Part model, mm, in its own coordinate system. Face numbers are marked on the shaded views. A direction names the side the tool comes from. Give positions to 0.01 mm unless a question says otherwise; leave off trailing zeros. Loops run counter-clockwise (first coordinate to the right, second up) from the corner with the lowest first, then second, coordinate; pieces in that order, holes last. Notation, with made-up numbers: (-27.75, 16.25) -> (-13.75, 16.25) arc R17 cw to (-13.75, 26.25) -> close; hole circle Ø4 at (-16.5, 81). An arc over 180 degrees is marked (long way). Write item = value, one per line.
from build123d import *

# Parameters (mm, degrees)
SKETCH1_W                                            = 110
SKETCH1_H                                            = 60
BOSS_EXTRUDE1_DEPTH                                  = 12
SKETCH2_R                                            = 12.5
CUT_EXTRUDE1_DEPTH                                   = 5
SKETCH3_R                                            = 10
CUT_EXTRUDE3_DEPTH                                   = 64.788713735
CHAMFER1_SIZE                                        = 3
M4_TAPPED_HOLE1_D                                    = 3.3
CBORE_FOR_M8_HEXAGON_SOCKET_HEAD_CAP_SCR_D           = 9
CBORE_FOR_M8_HEXAGON_SOCKET_HEAD_CAP_SCR_CBORE_D     = 15
CBORE_FOR_M8_HEXAGON_SOCKET_HEAD_CAP_SCR_CBORE_DEPTH = 9


with BuildPart() as part:
    # Sketch1 → Boss-Extrude1 (new body)
    with BuildSketch(Plane.XY):
        Rectangle(SKETCH1_W, SKETCH1_H)
    extrude(amount=BOSS_EXTRUDE1_DEPTH)

    # Sketch2 → Cut-Extrude1 (cut)
    with BuildSketch(Plane(origin=(0, 0, 12), x_dir=(-1, 0, 0), z_dir=(0, 0, -1))):
        with Locations((35, 0)):
            Circle(SKETCH2_R)
    extrude(amount=CUT_EXTRUDE1_DEPTH, mode=Mode.SUBTRACT)

    # Sketch3 → Cut-Extrude3 (cut, through all)
    with BuildSketch(Plane.XY.offset(12)):
        with Locations((-35, 0)):
            Circle(SKETCH3_R)
    extrude(amount=-CUT_EXTRUDE3_DEPTH, mode=Mode.SUBTRACT)

    # Chamfer1
    chamfer1_edges = [part.edges().sort_by_distance(p)[0] for p in [
        (55, -30, 6),
        (-55, -30, 6),
        (-55, 30, 6),
        (55, 30, 6),
    ]]
    chamfer(chamfer1_edges, length=CHAMFER1_SIZE)

    # M4 Tapped Hole1 (through all)
    with Locations(Plane.XY.offset(12)):
        with Locations((-35, 14.5), (-20.5, 0), (-49.5, 0), (-35, -14.5)):
            Hole(M4_TAPPED_HOLE1_D / 2)

    # CBORE for M8 Hexagon socket head cap screws1 (through all)
    with Locations(Plane(origin=(0, 0, 0), x_dir=(-1, 0, 0), z_dir=(0, 0, -1))):
        with Locations((-40, 15), (-40, -15)):
            CounterBoreHole(CBORE_FOR_M8_HEXAGON_SOCKET_HEAD_CAP_SCR_D / 2, CBORE_FOR_M8_HEXAGON_SOCKET_HEAD_CAP_SCR_CBORE_D / 2, CBORE_FOR_M8_HEXAGON_SOCKET_HEAD_CAP_SCR_CBORE_DEPTH)


solid = part.part
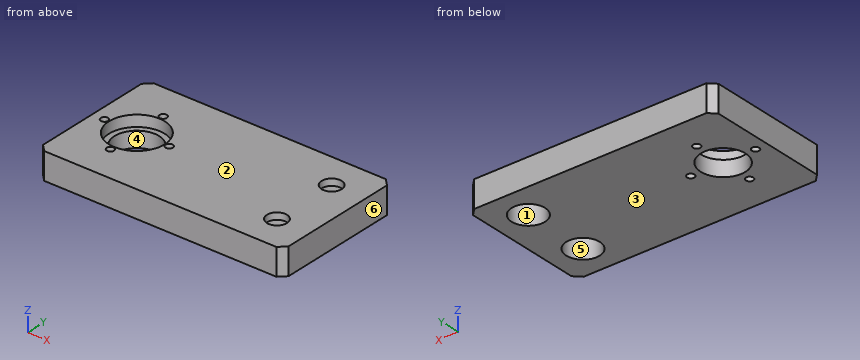
1) Slice it at C-C, the plane x = 42. List the corners of the cut face in (y, z).
Resolved:
outline = (-30, 0) -> (-22.23, 0) -> (-22.23, 9) -> (-19.03, 9) -> (-19.03, 12) -> (-30, 12) -> close; (-10.97, 9) -> (-7.77, 9) -> (-7.77, 0) -> (7.77, 0) -> (7.77, 9) -> (10.97, 9) -> (10.97, 12) -> (-10.97, 12) -> close; (19.03, 9) -> (22.23, 9) -> (22.23, 0) -> (30, 0) -> (30, 12) -> (19.03, 12) -> close
2) Drop flat-ended pins along their axis: P1, Ø4.5, axis at x = 38.5, y = 13, coming from the -Z side; P2, Ø5, axis at x = -32, y = 8.5, coming from the +Z side. Give the stop position or say it passes through.
Resolved:
P1 = 9
P2 = 7
3) Drill centre lines: line 1 along Y through (x, z) = (-35, 3); line 2 along Y through (x, z) = (-35, 11); line 3 along Y through (x, z) = (40, 3.5). Where is each one in solid material? Low to high. Write a range as [from, to].
Resolved:
line_1 = [-30, -16.15], [-12.85, -10], [10, 12.85], [16.15, 30]
line_2 = [-30, -16.15], [-12.85, -12.5], [12.5, 12.85], [16.15, 30]
line_3 = [-30, -22.5], [-7.5, 7.5], [22.5, 30]
4) Pull direction X, two halves, no side cores. Call the marked faces 3, 4, 5 and 6: pulls with the +X half, pulls with the -X half, needs draft (parallel to the pull), parting line crosses it, or undercut.
Resolved:
face_3 = needs draft
face_4 = undercut
face_5 = undercut
face_6 = pulls with the +X half
5) Slice it at A-A, the plane y = 0. List the corners of the cut face in (x, z), and give its area (3 significant figures).
Resolved:
outline = (-55, 0) -> (-51.15, 0) -> (-51.15, 12) -> (-55, 12) -> close; (-47.85, 0) -> (-45, 0) -> (-45, 7) -> (-47.5, 7) -> (-47.5, 12) -> (-47.85, 12) -> close; (-25, 0) -> (-22.15, 0) -> (-22.15, 12) -> (-22.5, 12) -> (-22.5, 7) -> (-25, 7) -> close; (-18.85, 0) -> (55, 0) -> (55, 12) -> (-18.85, 12) -> close
area = 976 mm²
6) Slice it at B-B, the plane x = -35. List the corners of the cut face in (y, z).
Resolved:
outline = (-30, 0) -> (-16.15, 0) -> (-16.15, 12) -> (-30, 12) -> close; (-12.85, 0) -> (-10, 0) -> (-10, 7) -> (-12.5, 7) -> (-12.5, 12) -> (-12.85, 12) -> close; (10, 0) -> (12.85, 0) -> (12.85, 12) -> (12.5, 12) -> (12.5, 7) -> (10, 7) -> close; (16.15, 0) -> (30, 0) -> (30, 12) -> (16.15, 12) -> close
7) Slice it at D-D, the plane y = -21. List the corners of the cut face in (x, z).
Resolved:
outline = (-55, 0) -> (35.5, 0) -> (35.5, 9) -> (44.5, 9) -> (44.5, 0) -> (55, 0) -> (55, 12) -> (-55, 12) -> close
8) Which spindle directions (+Z, -Z, +X, -X, +Y, -Y) get a long thin tool onto all of the face, cutting with end or side? Do the marked faces 1 and 2. Say none if no direction does.
Resolved:
face_1 = -Z
face_2 = +Z, +X, -X, +Y, -Y
